Can you work these out from the drawing? Everything is in mm from the part's minimum corner. A direction names the side the tool comes from. Give positions to 0.01 mm unless a question says otherwise; leave off trailing zeros. Write each loop counter-clockwise with the first axis right and the second up, starting at its lowest first coordinate (ties: lowest second). Pieces come first, ordered by that corner, then holes. Notation, with made-up numbers: (29, 25) -> (42, 25) arc R28 cw to (42, 61) -> close; hole circle Ø10 at (67.25, 8.5). An arc over 180 degrees is marked (long way). Use one line per item in the form item = value.
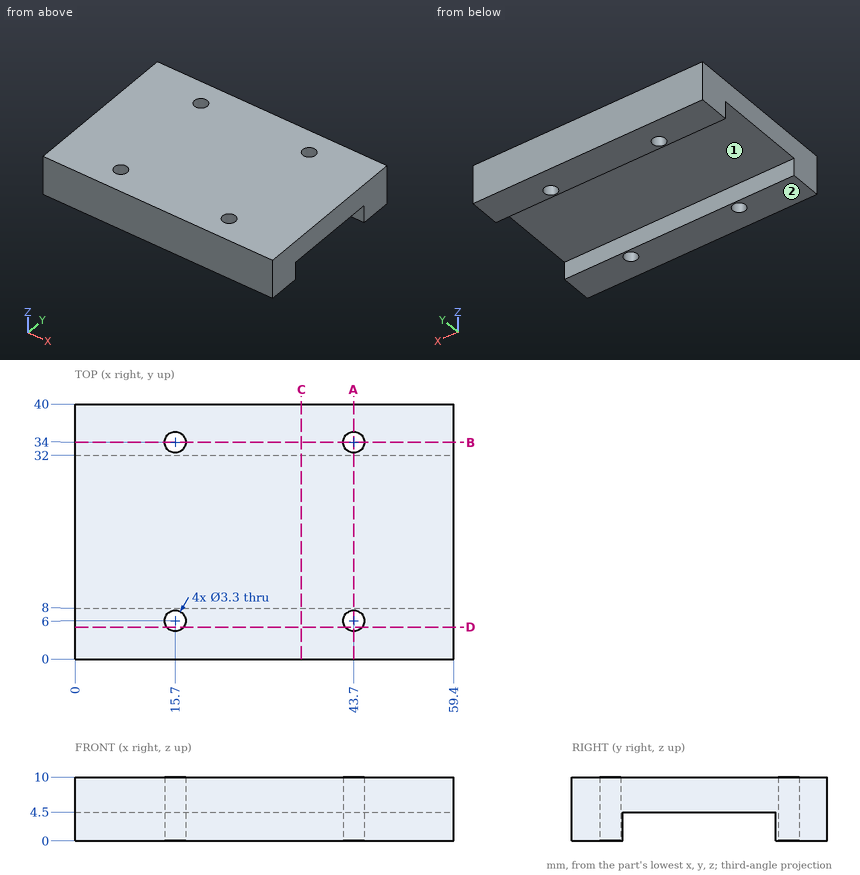
Q1. Which directions (+Z, -Z, +X, -X, +Y, -Y) give clear straight access to the entire face, cutting with the end or side of a thin tool? Please do the marked faces 1 and 2.
Result set:
face_1 = -Z, +X, -X
face_2 = -Z, +X, -X, +Y, -Y
Q2. I want a section at C-C, the plane x = 35.5. Write out the boundary of the cut face in (y, z), and give its area (3 significant figures).
Result set:
outline = (0, 0) -> (8, 0) -> (8, 4.5) -> (32, 4.5) -> (32, 0) -> (40, 0) -> (40, 10) -> (0, 10) -> close
area = 292 mm2
Q3. I want a section at A-A, the plane x = 43.7. Write out the boundary of the cut face in (y, z), and give its area (3 significant figures).
Result set:
outline = (0, 0) -> (4.35, 0) -> (4.35, 10) -> (0, 10) -> close; (7.65, 0) -> (8, 0) -> (8, 4.5) -> (32, 4.5) -> (32, 0) -> (32.35, 0) -> (32.35, 10) -> (7.65, 10) -> close; (35.65, 0) -> (40, 0) -> (40, 10) -> (35.65, 10) -> close
area = 226 mm2
Q4. I want a section at D-D, the plane y = 5. Write out the boundary of the cut face in (x, z).
Result set:
outline = (0, 0) -> (14.39, 0) -> (14.39, 10) -> (0, 10) -> close; (17.01, 0) -> (42.39, 0) -> (42.39, 10) -> (17.01, 10) -> close; (45.01, 0) -> (59.4, 0) -> (59.4, 10) -> (45.01, 10) -> close
Q5. If I drill on line 1 along Y through (x, z) = (15.7, 3.5); line 2 along Y through (x, z) = (15.7, 6.5); line 3 along Y through (x, z) = (33, 3.25), over which ranges is the centre line in solid material (lowest first)? Write a range as from..to.
Result set:
line_1 = 0..4.35, 7.65..8, 32..32.35, 35.65..40
line_2 = 0..4.35, 7.65..32.35, 35.65..40
line_3 = 0..8, 32..40
Q6. Will these pins go through, and if not, where does the flat tip stop? pin 1 Ø1.3 at (x, z) = (35, 1.5) entering from -Y; pin 2 Ø12 at (x, y) = (15, 19.5) entering from -Z.
Result set:
pin_1 = 0
pin_2 = 4.5
Q7. I want a section at B-B, the plane y = 34. Write out the boundary of the cut face in (x, z), and give its area (3 significant figures).
Result set:
outline = (0, 0) -> (14.05, 0) -> (14.05, 10) -> (0, 10) -> close; (17.35, 0) -> (42.05, 0) -> (42.05, 10) -> (17.35, 10) -> close; (45.35, 0) -> (59.4, 0) -> (59.4, 10) -> (45.35, 10) -> close
area = 528 mm2
